For this review, use the dimensioned drawing (mm, ordinates from the lowest corner) and the shaded views. Round coordinates to 2 decimals unless told otherwise and drop trailing zeros. Write each loop counter-clockwise with the first axis right and the second up, starting at its lowest first coordinate (ties: lowest second). Pieces come first, ordered by that corner, then holes. Notation, with made-up numbers: (-33, 46) -> (18, 46) arc R31 ccw to (18, 74) -> close; hole circle Ø1 at (50, 35). An arc over 180 degrees is marked (long way). Write each question's results on one line, items separated by ' | '. Start each with the question number.
Item 1: Add section C-C (z = 10). State the section outline as (x, y) points.
Item 2: Clearance check with flat-ended pins moving along their axes: pin 1 (22.5 mm diameter, centred on x = 50, y = 25, fed in from +Z); pin 2 (11 mm diameter, centred on x = 200, y = 195, fed in from +Z). State where each tip first meets the part, or that it passes through.
Item 3: Add section A-A (x = 200). State the section outline as (y, z) points, plus the area to 3 significant figures.
Item 4: To check wall thickness, follow line 1 along Y through (x, z) = (200, 8.75); line 2 along X through (y, z) = (23, 10.25); line 3 along X through (y, z) = (197.5, 12.5). State the ranges of each line that lie inside material, in increasing order.
Item 5: Add section B-B (y = 195). State the section outline as (x, z) points.
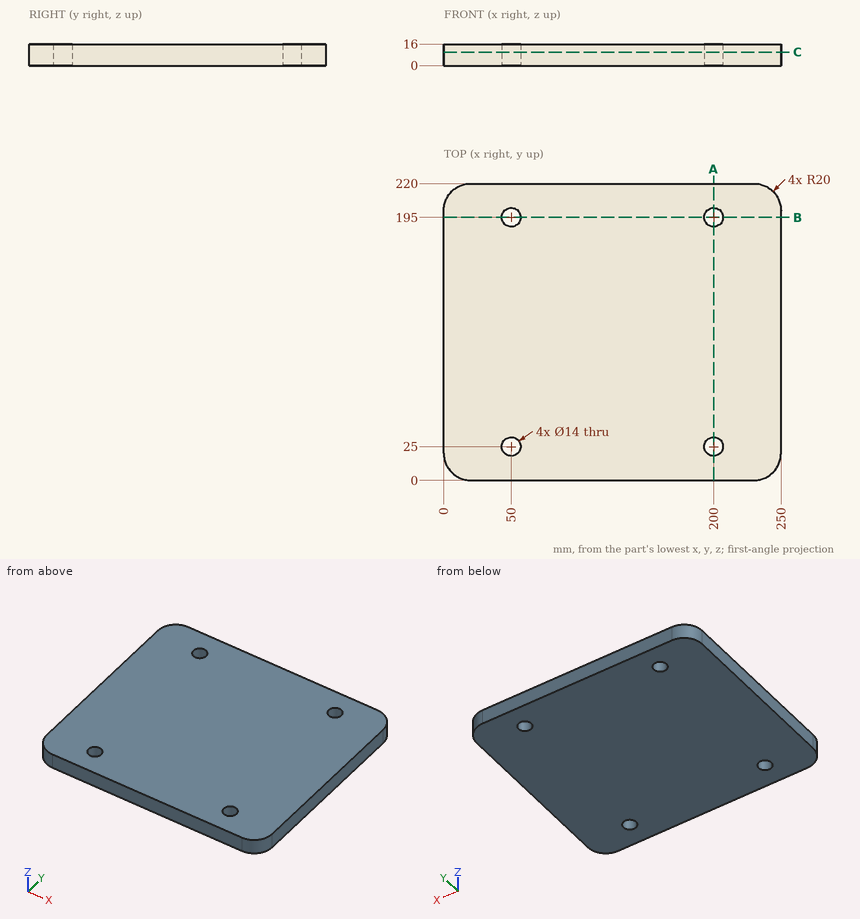
Responses:
1) outline: (0, 20) arc R20 ccw to (20, 0) -> (230, 0) arc R20 ccw to (250, 20) -> (250, 200) arc R20 ccw to (230, 220) -> (20, 220) arc R20 ccw to (0, 200) -> close; hole circle Ø14 at (50, 25); hole circle Ø14 at (50, 195); hole circle Ø14 at (200, 25); hole circle Ø14 at (200, 195)
2) pin 1: stops at z = 16 | pin 2: passes through
3) outline: (0, 0) -> (18, 0) -> (18, 16) -> (0, 16) -> close; (32, 0) -> (188, 0) -> (188, 16) -> (32, 16) -> close; (202, 0) -> (220, 0) -> (220, 16) -> (202, 16) -> close | area: 3,070 mm^2
4) line 1: y = 0 to 18, 32 to 188, 202 to 220 | line 2: x = 0 to 43.29, 56.71 to 193.29, 206.71 to 250 | line 3: x = 0 to 43.46, 56.54 to 193.46, 206.54 to 250
5) outline: (0, 0) -> (43, 0) -> (43, 16) -> (0, 16) -> close; (57, 0) -> (193, 0) -> (193, 16) -> (57, 16) -> close; (207, 0) -> (250, 0) -> (250, 16) -> (207, 16) -> close
